For this review, take the finished solid that the model builds, in its own axes (mm). Round coordinates to 2 decimals unless told otherwise and drop trailing zeros. Write each loop counter-clockwise with the first axis right and the second up, starting at its lowest first coordinate (ties: lowest second). Pieces come first, ordered by that corner, then holes. Notation, with made-up numbers: M 38.25,56 L 90.25,56 A6 cw 90.25,61 Z; hole C 84.25,68.5 d1. An arc over 180 degrees is marked long. One line per question, with ' | ' between items.
```python
from build123d import *

# Parameters (mm, degrees)
BOSS_EXTRUDE1_DEPTH = 310
SHELL1_T            = -2
CUT_EXTRUDE1_DEPTH  = 10
CUT_EXTRUDE2_DEPTH  = 397.026111511
CUT_EXTRUDE3_DEPTH  = 5
SKETCH5_R           = 3
CUT_EXTRUDE4_DEPTH  = 10
CUT_EXTRUDE5_DEPTH  = 397.026111511
CUT_EXTRUDE7_DEPTH  = 382.100397819
CUT_EXTRUDE8_DEPTH  = 211.562851919


with BuildPart() as part:
    # Sketch1 → Boss-Extrude1 (new body)
    with BuildSketch(Plane.XY):
        Polygon((-174.265144247, 0), (-123.224065222, -123.224065222), (0, -174.265144247), (123.224065222, -123.224065222), (174.265144247, 0), (123.224065222, 123.224065222), (0, 174.265144247), (-123.224065222, 123.224065222), align=None)
    extrude(amount=BOSS_EXTRUDE1_DEPTH)

    # Shell1
    shell1_openings = [part.faces().sort_by_distance(p)[0] for p in [
        (0, 0, 0),
    ]]
    offset(amount=SHELL1_T, openings=shell1_openings, kind=Kind.INTERSECTION)

    # Sketch2 → Cut-Extrude1 (cut)
    with BuildSketch(Plane.XY.offset(310)):
        Polygon((104.089893603, 104.089893603), (0, 147.20533924), (-104.089893603, 104.089893603), (-147.20533924, 0), (-104.089893603, -104.089893603), (0, -147.20533924), (104.089893603, -104.089893603), (147.20533924, 0), align=None)
    extrude(amount=-CUT_EXTRUDE1_DEPTH, mode=Mode.SUBTRACT)

    # Sketch3 → Cut-Extrude2 (cut, through all)
    with BuildSketch(Plane.XY.offset(310)):
        Polygon((70.138181093, 169.328548035), (-63.801020235, -154.029288344), (130.028007017, -234.315900213), (263.967208344, 89.041936166), align=None)
    extrude(amount=-CUT_EXTRUDE2_DEPTH, mode=Mode.SUBTRACT)

    # Sketch4 → Cut-Extrude3 (cut)
    with BuildSketch(Plane.XY.offset(310)):
        Polygon((-143.932898959, 151.622295845), (-51.544945707, 113.353952609), (-116.60112921, -43.705567918), (-208.989082461, -5.437224682), align=None)
    extrude(amount=-CUT_EXTRUDE3_DEPTH, mode=Mode.SUBTRACT)

    # Sketch5 → Cut-Extrude4 (cut)
    with BuildSketch(Plane.XY.offset(310)):
        with Locations((0, 155.323280742)):
            Circle(SKETCH5_R)
        with Locations((-46.193976626, 136.189109124)):
            Circle(SKETCH5_R)
        with Locations((46.193976626, 136.189109124)):
            Circle(SKETCH5_R)
        with Locations((-128.964316707, -63.636168463)):
            Circle(SKETCH5_R)
        with Locations((-109.830145089, -109.830145089)):
            Circle(SKETCH5_R)
        with Locations((-63.636168463, -128.964316707)):
            Circle(SKETCH5_R)
    extrude(amount=-CUT_EXTRUDE4_DEPTH, mode=Mode.SUBTRACT)

    # Sketch19 → Cut-Extrude5 (cut, through all)
    with BuildSketch(Plane.XY.offset(310)):
        Polygon((-32.528091751, -78.529760263), (61.612032611, 148.744604734), (-87.132572124, 210.356637345), (-181.272696485, -16.917727653), align=None)
    extrude(amount=-CUT_EXTRUDE5_DEPTH, mode=Mode.SUBTRACT)

    # Sketch21 → Cut-Extrude7 (cut, through all)
    with BuildSketch(Plane.XY.offset(310)):
        Polygon((-117.866497168, -117.866497168), (-58.933248584, -142.277448007), (-61.612032611, -148.744604734), (-123.224065222, -123.224065222), (-164.354968833, -23.925279891), (-155.209028079, -27.713652592), align=None)
    extrude(amount=-CUT_EXTRUDE7_DEPTH, mode=Mode.SUBTRACT)

    # Sketch22 → Cut-Extrude8 (cut, through all)
    with BuildSketch(Plane.XY.offset(310)):
        Polygon((-154.060977781, -30.48529119), (-155.209028079, -27.713652592), (-151.289339184, -29.337240892), align=None)
    extrude(amount=-CUT_EXTRUDE8_DEPTH, mode=Mode.SUBTRACT)


solid = part.part
```
Item 1: Mouldability with a two-part tool opening along Y and no side actions: class faces 1 (the face through (-131.175, -61.609, 309.014)), 2 (the face through (-118.08, -70.31, 309.01)), 3 (the face through (-111, -90, 310)) as +Y half, -Y half, draft (parallel to the pull), parting line (faces both ways), or undercut.
Results:
face 1: undercut | face 2: +Y half | face 3: draft
Item 2: To check wall thickness, follow line 1 along Y through (x, z) = (-129.5, 308.55); line 2 along X through (y, z) = (-131.5, 309.45); line 3 along X through (y, z) = (-109, 309.75). State the ranges of each line that lie inside material, in increasing order. Write a range as from..to.
Results:
line 1: -89.78..-66.59, -60.68..-42.74 | line 2: -84.95..-65.24, -62.03..-54.47 | line 3: -121.54..-112.71, -106.95..-92.24
Item 3: Take a section at B-B (z = 309.6). Write out the cut boundary in (x, y).
Results:
outline: M -154.06,-30.49 L -117.87,-117.87 L -58.93,-142.28 L -52.04,-125.65 L -104.09,-104.09 L -131.69,-37.46 L -151.29,-29.34 Z; hole C -128.96,-63.64 d6; hole C -109.83,-109.83 d6; hole C -63.64,-128.96 d6
Item 4: Insertion check: pin 1 Ø5 at (x, y) = (-63.64, -128.96) entering from +Z. The pin has a flat end and moves straight along its axis. Give the tip position at first contact, or say it passes through.
Results:
pin 1: through
Item 5: Take a section at D-D (x = -81.5). Write out the cut boundary in (y, z).
Results:
outline: M -132.93,308 L -113.45,308 L -113.45,310 L -132.93,310 Z
Item 6: Take a section at C-C (y = -135). Write out the cut boundary in (x, z), then the cut area to 3 significant figures.
Results:
outline: M -76.5,308 L -55.92,308 L -55.92,310 L -76.5,310 Z | area: 41.2 mm2
Item 7: Take a section at A-A (x = -130). Write out the cut boundary in (y, z).
Results:
outline: M -88.57,308 L -66.45,308 L -66.45,310 L -88.57,310 Z; M -60.82,308 L -41.54,308 L -41.54,310 L -60.82,310 Z
